The drawing under review shows one solid part. Ordinate dimensions are in mm from its lowest x, y, z. A direction names the side the tool comes from. Round coordinates to 2 decimals unless told otherwise and drop trailing zeros. Loops run counter-clockwise (first coordinate to the right, second up) from the corner with the lowest first, then second, coordinate; pieces in that order, holes last. Notation, with made-up numbers: (-36.75, 21.25) -> (-17.75, 21.25) arc R21 ccw to (-17.75, 36.25) -> close; hole circle Ø6 at (87.5, 89.25). An arc over 180 degrees is marked (long way). Answer as CSV lines item,"result". Start each with the question number.
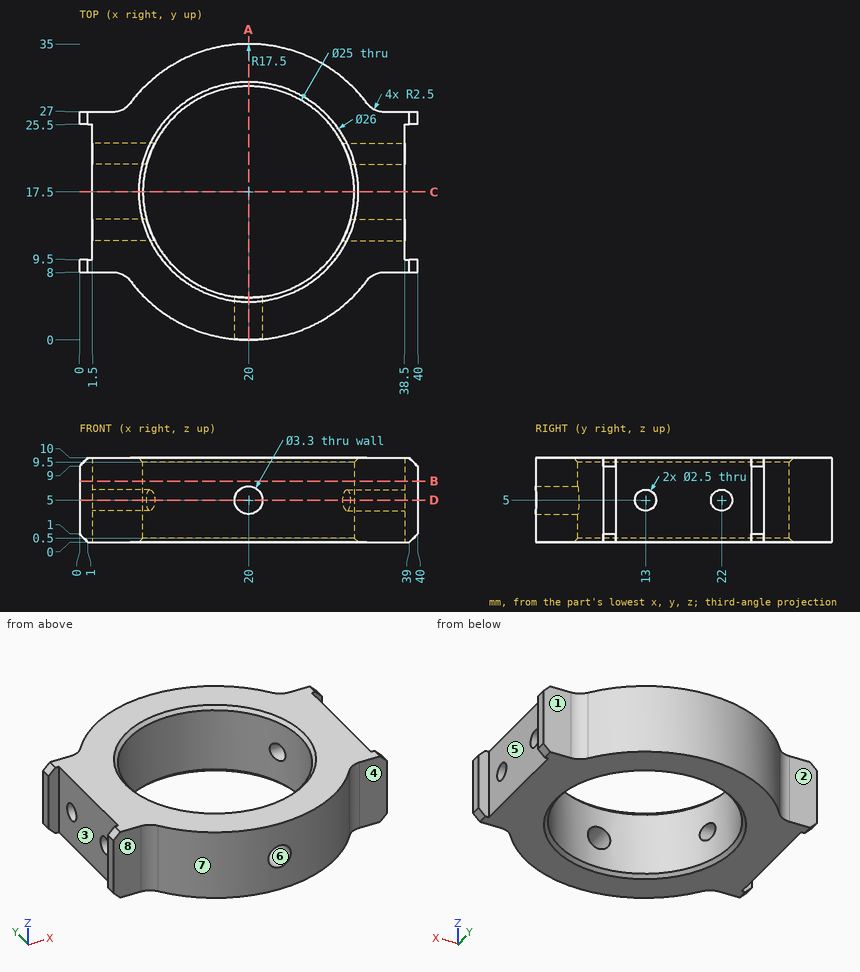
Q1. To check wall thickness, follow probe 1 along Y at (x, z) = (5, 5); probe 2 along Y at (x, z) = (35.5, 5); probe 3 along X at (y, z) = (25, 5.5). State the ranges of each line that lie inside material, in increasing order. Write a range as from..to.
Q2. Add section A-A, the plane x = 20. Give the boundary of the cut face in (y, z).
Q3. For pin 1 Ø1.2 at (x, z) = (39.5, 3.5) entering from +Y; pin 2 Ø1.2 at (x, z) = (1, 5) entering from -Y; pin 3 Ø4.5 at (x, z) = (2.5, 4) entering from -Y, all flat-tipped, find the tip position at first contact; note any pin that passes through.
Q4. Add section D-D, the plane z = 5. State how many separate pieces and enclosed holes the cut face has, and give its area (3 significant figures).
Q5. Add section B-B, the plane z = 7.25. Give the boundary of the cut face in (x, y).
Q6. Machinability: for the marked faces 1, 2, 3, 4 and 5, which of the approach directions +Z, -Z, +X, -X, +Y, -Y give a long, thin tool a straight path to every point of the face, cutting with its end or side? Answer none if there is none.
Q7. Mouldability with a two-part tool opening along X and no side actions: class the marked faces 6, 7 and 8 as pulls with the +X half, pulls with the -X half, needs draft (parallel to the pull), parting line crosses it, or undercut.
Q8. Add section C-C, the plane y = 17.5. Give the boundary of the cut face in (x, z).
Worked answers:
1,probe 1,"y = 7.79..11.75, 14.25..20.75, 23.25..27.21"
1,probe 2,"y = 7.95..11.75, 14.25..20.75, 23.25..27.05"
1,probe 3,"x = 1.5..10, 30..38.5"
2,outline,"(0, 0) -> (4.5, 0) -> (5, 0.5) -> (5, 3.35) -> (0, 3.35) -> close; (0, 6.65) -> (5, 6.65) -> (5, 9.5) -> (4.5, 10) -> (0, 10) -> close; (30, 0.5) -> (30.5, 0) -> (35, 0) -> (35, 10) -> (30.5, 10) -> (30, 9.5) -> close"
3,pin 1,"stops at y = 27"
3,pin 2,"stops at y = 8"
3,pin 3,"stops at y = 7.88"
4,separate pieces,"5"
4,enclosed holes,"0"
4,area,"468 mm^2"
5,outline,"(0, 8) -> (4, 8) arc R2.5 cw to (6, 7) arc R17.5 ccw to (34, 7) arc R2.5 cw to (36, 8) -> (40, 8) -> (40, 9.5) -> (38.5, 9.5) -> (38.5, 25.5) -> (40, 25.5) -> (40, 27) -> (36, 27) arc R2.5 cw to (34, 28) arc R17.5 ccw to (6, 28) arc R2.5 cw to (4, 27) -> (0, 27) -> (0, 25.5) -> (1.5, 25.5) -> (1.5, 9.5) -> (0, 9.5) -> close; hole circle Ø25 at (20, 17.5)"
6,face 1,"+Z, -Z, +X, +Y"
6,face 2,"+Z, -Z, -X, +Y"
6,face 3,"+Z, -Z, -X"
6,face 4,"+Z, -Z, +X, -Y"
6,face 5,"+Z, -Z, +X"
7,face 6,"undercut"
7,face 7,"parting line crosses it"
7,face 8,"needs draft"
8,outline,"(1.5, 0) -> (7, 0) -> (7.5, 0.5) -> (7.5, 9.5) -> (7, 10) -> (1.5, 10) -> close; (32.5, 0.5) -> (33, 0) -> (38.5, 0) -> (38.5, 10) -> (33, 10) -> (32.5, 9.5) -> close"
